Geometry: final body of the model. Coordinates: model frame, mm. Face numbers are marked on the shaded views. A direction names the side the tool comes from. Round coordinates to 2 decimals unless told otherwise and drop trailing zeros. Loops run counter-clockwise (first coordinate to the right, second up) from the corner with the lowest first, then second, coordinate; pieces in that order, holes last. Notation, with made-up numbers: (-10, 57.25) - (-2, 57.25) arc R8 cw to (-2, 72.25) - close; hole circle Ø11 at (58.5, 58). An arc over 180 degrees is marked (long way). Use CSV: the item, a comma, the result in double quotes.
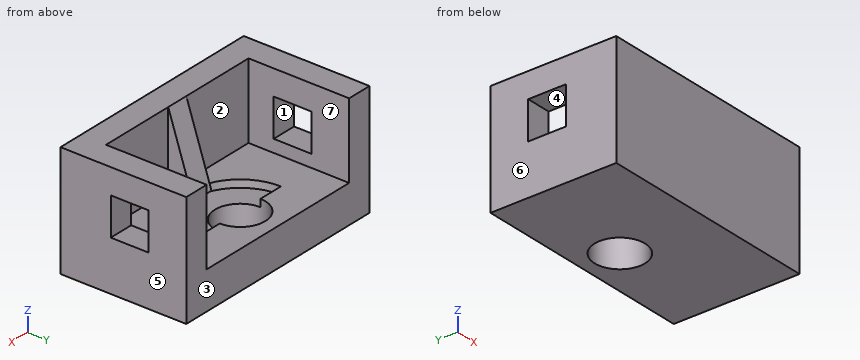
from build123d import *

# Parameters (mm, degrees)
BLOCK_PROFILE_SKETCH_90X50_W   = 90
BLOCK_PROFILE_SKETCH_90X50_H   = 50
BASE_BLOCK_90X50X45_DEPTH      = 45
POCKET_SKETCH_W                = 70
POCKET_SKETCH_H                = 40
INNER_POCKET_30_DEEP_DEPTH     = 30
BORE_SKETCH_R                  = 10
GUIDE_BORE_CUT_DEPTH           = 60.581876439
SIDE_WINDOW_SKETCH_W           = 15
SIDE_WINDOW_SKETCH_H           = 15
SIDE_WINDOWS_15X15_DEPTH       = 104.682206767
RIB_SKETCH_W                   = 8.881329336
RIB_SKETCH_H                   = 10
INTERNAL_RIB_DEPTH             = 30
ARC_RELIEF_GROOVE_3_DEEP_DEPTH = 3
RIB_TRIM_CUT_10_DEEP_DEPTH     = 10


with BuildPart() as part:
    # Block Profile Sketch 90x50 → Base Block 90x50x45 (new body)
    with BuildSketch(Plane.XY):
        Rectangle(BLOCK_PROFILE_SKETCH_90X50_W, BLOCK_PROFILE_SKETCH_90X50_H)
    extrude(amount=-BASE_BLOCK_90X50X45_DEPTH)

    # Pocket Sketch → Inner Pocket 30 Deep (cut)
    with BuildSketch(Plane.XY):
        with Locations((0, 5)):
            Rectangle(POCKET_SKETCH_W, POCKET_SKETCH_H)
    extrude(amount=-INNER_POCKET_30_DEEP_DEPTH, mode=Mode.SUBTRACT)

    # Bore Sketch → Guide Bore Cut (cut, through all)
    with BuildSketch(Plane.XY.offset(-30)):
        with Locations((0, 10)):
            Circle(BORE_SKETCH_R)
    extrude(amount=-GUIDE_BORE_CUT_DEPTH, mode=Mode.SUBTRACT)

    # Side Window Sketch → Side Windows 15x15 (cut, through all)
    with BuildSketch(Plane.ZY.offset(45)):
        with Locations((-17.5, 2.5)):
            Rectangle(SIDE_WINDOW_SKETCH_W, SIDE_WINDOW_SKETCH_H)
    extrude(amount=-SIDE_WINDOWS_15X15_DEPTH, mode=Mode.SUBTRACT)

    # Rib Sketch → Internal Rib (add)
    with BuildSketch(Plane.XY.offset(-30)):
        with Locations((0, -10)):
            Rectangle(RIB_SKETCH_W, RIB_SKETCH_H)
    extrude(amount=INTERNAL_RIB_DEPTH)

    # Arc Groove Sketch → Arc Relief Groove 3 Deep (cut)
    with BuildSketch(Plane.XY.offset(-30)):
        with BuildLine():
            Line((20, 10), (10, 10))
            ThreePointArc((10, 10), (0, 0), (-10, 10))
            Line((-10, 10), (-20, 10))
            ThreePointArc((-20, 10), (0, -10), (20, 10))
        make_face()
    extrude(amount=-ARC_RELIEF_GROOVE_3_DEEP_DEPTH, mode=Mode.SUBTRACT)

    # Rib Trim Sketch → Rib Trim Cut 10 Deep (cut)
    with BuildSketch(Plane(origin=(4.440664668, 0, 0), x_dir=(0, 0, -1), z_dir=(1, 0, 0))):
        Polygon((30, -5), (0, -5), (0, -15), align=None)
    extrude(amount=-RIB_TRIM_CUT_10_DEEP_DEPTH, mode=Mode.SUBTRACT)


solid = part.part
Item 1: Reachability of the marked faces 1, 2 and 3 from +Z, -Z, +X, -X, +Y, -Y: full face, straight path, thin tool, end or side. Return the list, or none.
Final values:
face 1,"+X, -X"
face 2,"+Z, +Y"
face 3,"+Z, -Z, +X, -X, +Y"
Item 2: Section B-B on x = 0. Return the cut outline in (y, z).
Final values:
outline,"(-25, -45) - (0, -45) - (0, -33) - (-10, -33) - (-10, -30) - (-5, -30) - (-15, 0) - (-25, 0) - close; (20, -45) - (25, -45) - (25, -30) - (20, -30) - close"
Item 3: Pin query (flat end, axial travel): P1, Ø3, axis at x = 31.5, z = -10.5, coming from the +Y side; P2, Ø8, axis at x = 22.5, y = -6.5, coming from the +Z side. Return the tip coordinate at first contact, or that it passes through.
Final values:
P1,"stops at y = -15"
P2,"stops at z = -30"
Item 4: Section D-D on x = 36. Return the cut outline in (y, z).
Final values:
outline,"(-25, -45) - (25, -45) - (25, 0) - (-25, 0) - close; hole (-5, -25) - (10, -25) - (10, -10) - (-5, -10) - close"
Item 5: Material intervals for line 1 (Y direction, x = 0, z = -41.75); line 2 (X direction, y = 9.5, z = -3.5); line 3 (X direction, y = 10, z = -36), sorted ascending.
Final values:
line 1,"y = -25 to 0, 20 to 25"
line 2,"x = -45 to -35, 35 to 45"
line 3,"x = -45 to -10, 10 to 45"
Item 6: Section C-C on z = -31. Return the cut outline in (x, y).
Final values:
outline,"(-45, -25) - (45, -25) - (45, 25) - (-45, 25) - close; hole (-20, 10) arc R20 ccw to (20, 10) - (10, 10) arc R10 ccw to (-10, 10) - close"
Item 7: Mould query, pull axis X, two halves, no side actions, for the marked faces 4, 5, 6 and 7. Classes: released by +X, released by -X, zero draft, split by the parting line, or undercut.
Final values:
face 4,"zero draft"
face 5,"released by +X"
face 6,"released by -X"
face 7,"undercut"
Item 8: Section A-A on z = -15. Return the cut outline in (x, y).
Final values:
outline,"(-45, -25) - (45, -25) - (45, -5) - (35, -5) - (35, -15) - (4.44, -15) - (4.44, -10) - (-4.44, -10) - (-4.44, -15) - (-35, -15) - (-35, -5) - (-45, -5) - close; (-45, 10) - (-35, 10) - (-35, 25) - (-45, 25) - close; (35, 10) - (45, 10) - (45, 25) - (35, 25) - close"
